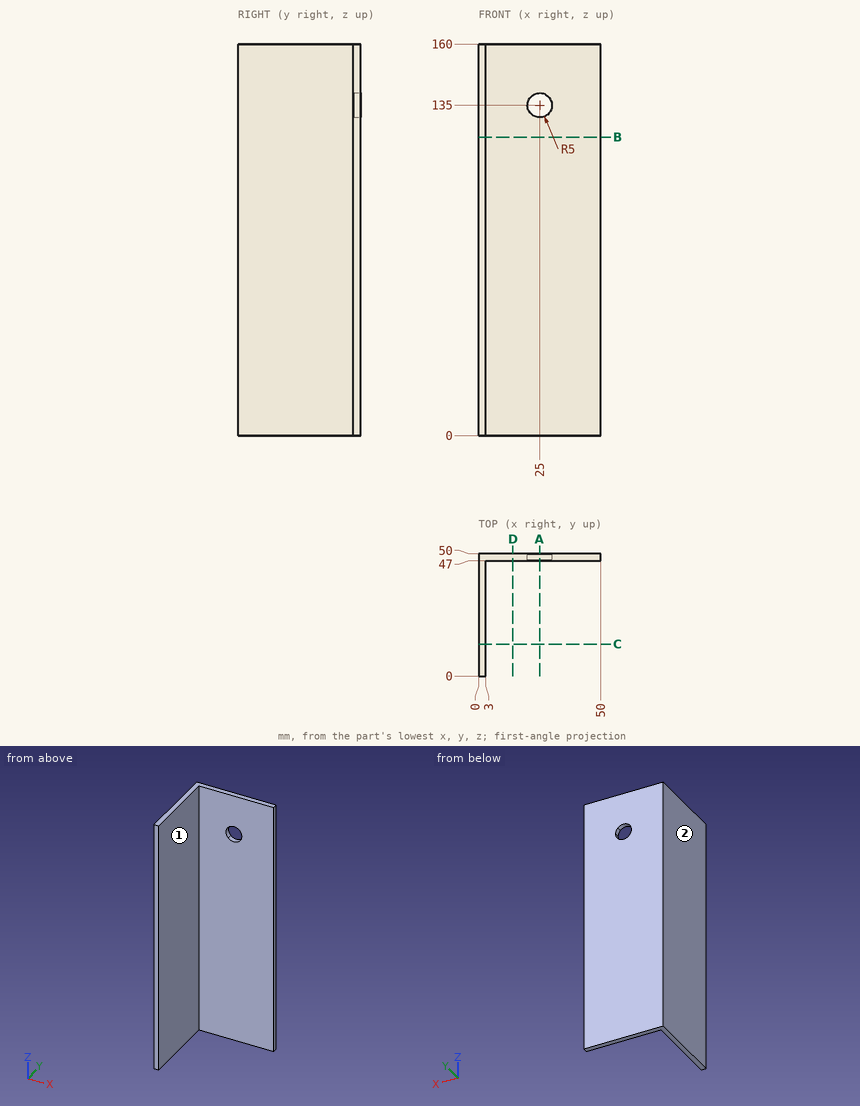
Study the drawing (mm; zero at the part's minimum x, y, z) and answer. A direction names the side the tool comes from. Coordinates: 2 decimals unless noted, no trailing zeros. Write each loop counter-clockwise with the first axis right and the second up, starting at its lowest first coordinate (ties: lowest second). Pieces come first, ordered by that corner, then holes. Notation, with made-up numbers: (-36, 89) - (-16, 89) arc R17 ccw to (-16, 103) - close; hole circle Ø9 at (20.25, 45). An arc over 180 degrees is marked (long way). Return JSON: item names as keys, results as strings. Group by question number.
1. A cutting plane is placed at A-A, the plane x = 25. Determine the outline of the cut face in (y, z), plus the area to 3 significant figures.
2. A cutting plane is placed at B-B, the plane z = 122. Determine the outline of the cut face in (x, y).
3. A cutting plane is placed at C-C, the plane y = 13. Determine the outline of the cut face in (x, z).
4. Straight lines are drawn through the part: L1, parallel to X at y = 43.5, z = 139.5; L2, parallel to Y at x = 31.5, z = 123.5. For each, find the intervals that lie inside material, in ascending order.
5. A cutting plane is placed at D-D, the plane x = 14. Determine the outline of the cut face in (y, z), plus the area to 3 significant figures.
6. Which of the six approach directions +Z, -Z, +X, -X, +Y, -Y give full straight-line access (tool end or side, diameter ignored) to the marked faces 1 and 2?
7. Given pin 1 (1.5 mm diameter, centred on y = 14, z = 88, fed in from +X); pin 2 (5 mm diameter, centred on y = 11, z = 142, fed in from -X); pin 3 (1.5 mm diameter, centred on x = 6.5, z = 101.5, fed in from -Y), each flat-ended and moving along its own axis, determine where each tip first touches the part or whether it passes through.
Ans:
{
 "1": {"outline": "(47, 0) - (50, 0) - (50, 130) - (47, 130) - close; (47, 140) - (50, 140) - (50, 160) - (47, 160) - close", "area": "450 mm²"},
 "2": {"outline": "(0, 0) - (3, 0) - (3, 47) - (50, 47) - (50, 50) - (0, 50) - close"},
 "3": {"outline": "(0, 0) - (3, 0) - (3, 160) - (0, 160) - close"},
 "4": {"L1": "0 to 3", "L2": "47 to 50"},
 "5": {"outline": "(47, 0) - (50, 0) - (50, 160) - (47, 160) - close", "area": "480 mm²"},
 "6": {"face 1": "+Z, -Z, +X, -Y", "face 2": "+Z, -Z, -X, +Y, -Y"},
 "7": {"pin 1": "x = 3", "pin 2": "x = 0", "pin 3": "y = 47"}
}
